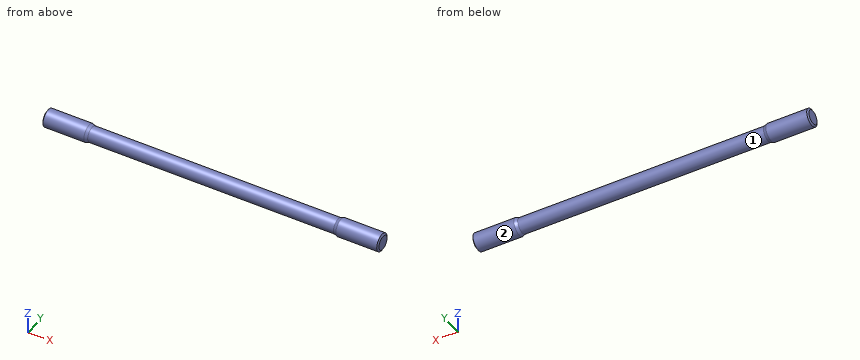
from build123d import *


with BuildPart() as part:
    # 草图1 → Revolve 558 (revolve)
    with BuildSketch(Plane.XY, mode=Mode.PRIVATE) as revolve_558_sk:
        Polygon((-152, 8), (-114, 8), (-111.2, 6.928), (111.2, 6.928), (114, 8), (152, 8), (152, 0), (-152, 0), align=None)
    revolve(revolve_558_sk.sketch.rotate(Axis((-152, 0, 0), (1, 0, 0)), 180), axis=Axis((-152, 0, 0), (1, 0, 0)))

    # 草图2 → Cut-Revolve 607 (revolve, cut)
    with BuildSketch(Plane.XY, mode=Mode.PRIVATE) as cut_revolve_607_sk:
        Polygon((-152.999970666, 8), (-151.000029334, 8), (-152, 6.268), align=None)
    cut_revolve_607 = revolve(cut_revolve_607_sk.sketch.rotate(Axis((-26.952426469, 0, 0), (1, 0, 0)), 180), axis=Axis((-26.952426469, 0, 0), (1, 0, 0)), mode=Mode.SUBTRACT)

    # 镜向1: Cut-Revolve 607 across plane
    add(cut_revolve_607.mirror(Plane(origin=(0, 0, 0), x_dir=(0, 0, 1), z_dir=(1, 0, 0))), mode=Mode.SUBTRACT)


solid = part.part
Here's how the part is built. I have some questions about the finished solid (model axes, mm). Face numbers are marked on the shaded views. Round coordinates to 2 decimals unless told otherwise and drop trailing zeros. Loops run counter-clockwise (first coordinate to the right, second up) from the corner with the lowest first, then second, coordinate; pieces in that order, holes last. Notation, with made-up numbers: M 21.5,-19 L 38.5,-19 A25 ccw 38.5,4 Z; hole C 74,38.25 d4. An arc over 180 degrees is marked long. Write each question's results on one line, items separated by ' | '. Start each with the question number.
(1) Thinking about a two-plate mould opening in X: for the marked faces 1 and 2, which applies, pulls with the +X half, pulls with the -X half, needs draft (parallel to the pull), parting line crosses it, or undercut?
(2) If I drill on probe 1 along Y at (x, z) = (-49, -0.5); probe 2 along Z at (x, y) = (-41, -3); probe 3 along Z at (x, y) = (-48, -4.25), over which ranges is the centre line in solid material (lowest first)? Write a range as from..to.
(3) I want a section at C-C (x = 22.5). Please give me the cut outline in (y, z), then the cut area to 3 significant figures.
(4) Will these pins go through, and if not, where does the flat tip stop? P1, Ø8, axis at x = -52.5, z = 3.5, coming from the +Y side; P2, Ø1, axis at x = -116.5, y = -5, coming from the -Z side; P3, Ø4, axis at x = -0.5, z = -4, coming from the -Y side; P4, Ø1.5, axis at y = -2.5, z = -6, coming from the -X side.
(5) I want a section at A-A (z = 0). Please give me the cut outline in (x, y).
Solved:
1) face 1: undercut | face 2: needs draft
2) probe 1: y = -6.91..6.91 | probe 2: z = -6.24..6.24 | probe 3: z = -5.47..5.47
3) outline: C 0,0 d13.86 | area: 151 mm²
4) P1: stops at y = 6.93 | P2: stops at z = -6.61 | P3: stops at y = -6.63 | P4: stops at x = -152
5) outline: M -152,-6.27 L -151,-8 L -114,-8 L -111.2,-6.93 L 111.2,-6.93 L 114,-8 L 151,-8 L 152,-6.27 L 152,6.27 L 151,8 L 114,8 L 111.2,6.93 L -111.2,6.93 L -114,8 L -151,8 L -152,6.27 Z
